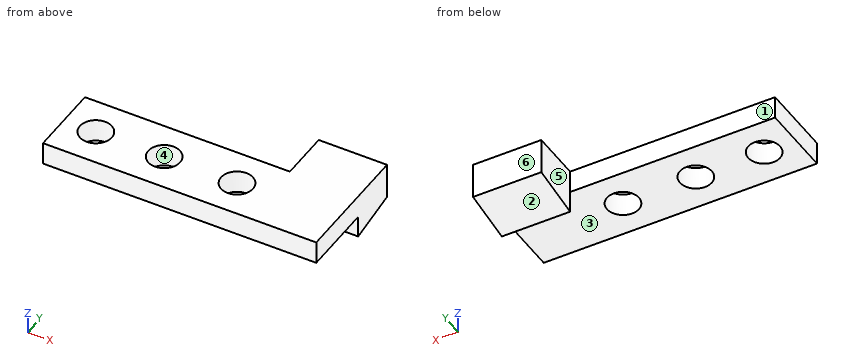
from build123d import *

# Parameters (mm, degrees)
BOSS_EXTRUDE1_DEPTH = 60
SKETCH2_W           = 45
SKETCH2_H           = 11
CUT_EXTRUDE1_DEPTH  = 60
SKETCH3_R           = 3.5
CUT_EXTRUDE2_DEPTH  = 60


with BuildPart() as part:
    # Sketch1 → Boss-Extrude1 (new body)
    with BuildSketch(Plane(origin=(0, 0, 0), x_dir=(0, 0, -1), z_dir=(1, 0, 0))):
        Polygon((0, 0), (0, 27), (7.89031, 27), (9.829906784, 16), (5, 16), (5, 0), align=None)
    extrude(amount=BOSS_EXTRUDE1_DEPTH)

    # Sketch2 → Cut-Extrude1 (cut)
    with BuildSketch(Plane.XY):
        with Locations((22.5, 21.5)):
            Rectangle(SKETCH2_W, SKETCH2_H)
    extrude(amount=-CUT_EXTRUDE1_DEPTH, mode=Mode.SUBTRACT)

    # Sketch3 → Cut-Extrude2 (cut)
    with BuildSketch(Plane.XY):
        with Locations((7, 8)):
            Circle(SKETCH3_R)
        with Locations((22, 8)):
            Circle(SKETCH3_R)
        with Locations((38, 8)):
            Circle(SKETCH3_R)
    extrude(amount=-CUT_EXTRUDE2_DEPTH, mode=Mode.SUBTRACT)


solid = part.part
Geometry check sheet. Reference: the model listing, model coordinates, mm. Face numbers are marked on the shaded views. A direction names the side the tool comes from. Round coordinates to 2 decimals unless told otherwise and drop trailing zeros. Write each loop counter-clockwise with the first axis right and the second up, starting at its lowest first coordinate (ties: lowest second). Pieces come first, ordered by that corner, then holes. Notation, with made-up numbers: (27.5, 23.25) -> (58.5, 23.25) arc R25 cw to (58.5, 53.25) -> close; hole circle Ø2 at (25.25, 1.5). An arc over 180 degrees is marked (long way). One line per item, written item: value. Start each with the question number.
(1) Draft check along X on the marked faces 4, 5 and 6. Enter one of: +X half, -X half, draft (parallel to the pull), parting line (faces both ways), or undercut.
(2) Cross-section at B-B, the plane x = 38. Record the cut outline in (y, z).
(3) Cross-section at A-A, the plane y = 8. Record the cut outline in (x, z).
(4) Cross-section at D-D, the plane x = 56.5. Record the cut outline in (y, z), and give its area (3 significant figures).
(5) Go/stop test with flat-tipped pins: pin 1 Ø10 at (x, y) = (54, 4.5) entering from -Z; pin 2 Ø1 at (y, z) = (23, -1.5) entering from -X; pin 3 Ø4 at (x, z) = (15.5, -3) entering from +Y. Record where each tip stops, or that it passes through.
(6) Cross-section at C-C, the plane z = -2.5. Record the cut outline in (x, y), and give its area (3 significant figures).
(7) Scan lines: line 1 (Y direction, x = 22, z = -2.35); line 2 (X direction, y = 10.75, z = -4.5); line 3 (Z direction, x = 26, y = 13.5). Record each from-to range of solid material in increasing order. Write a range as [from, to].
(8) Access from +Z, -Z, +X, -X, +Y, -Y to the whole of each face (thin tool, end or side, straight path). Record for the marked faces 1, 2 and 3.
Answer:
1. face 4: undercut
1. face 5: -X half
1. face 6: draft
2. outline: (0, -5) -> (4.5, -5) -> (4.5, 0) -> (0, 0) -> close; (11.5, -5) -> (16, -5) -> (16, 0) -> (11.5, 0) -> close
3. outline: (0, -5) -> (3.5, -5) -> (3.5, 0) -> (0, 0) -> close; (10.5, -5) -> (18.5, -5) -> (18.5, 0) -> (10.5, 0) -> close; (25.5, -5) -> (34.5, -5) -> (34.5, 0) -> (25.5, 0) -> close; (41.5, -5) -> (60, -5) -> (60, 0) -> (41.5, 0) -> close
4. outline: (0, -5) -> (16, -5) -> (16, -9.83) -> (27, -7.89) -> (27, 0) -> (0, 0) -> close
4. area: 177 mm²
5. pin 1: z = -5
5. pin 2: x = 45
5. pin 3: y = 16
6. outline: (0, 0) -> (60, 0) -> (60, 27) -> (45, 27) -> (45, 16) -> (0, 16) -> close; hole circle Ø7 at (7, 8); hole circle Ø7 at (22, 8); hole circle Ø7 at (38, 8)
6. area: 1,010 mm²
7. line 1: [0, 4.5], [11.5, 16]
7. line 2: [0, 4.83], [9.17, 19.83], [24.17, 35.83], [40.17, 60]
7. line 3: [-5, 0]
8. face 1: +Z, -Z, -X, +Y
8. face 2: -Z, +X, -X, +Y
8. face 3: -Z, +X, -X, -Y
